Check sheet for the modelled part. Datum: model origin and axes. Units: mm. Face numbers are marked on the shaded views. A direction names the side the tool comes from. Give positions to 0.01 mm unless a question says otherwise; leave off trailing zeros. Loops run counter-clockwise (first coordinate to the right, second up) from the corner with the lowest first, then second, coordinate; pieces in that order, holes last. Notation, with made-up numbers: M 82,58.25 L 117,58.25 A26 cw 117,95.25 Z; hole C -7.75,-9.5 d10. An arc over 180 degrees is marked long. Use one line per item in the form item = value.
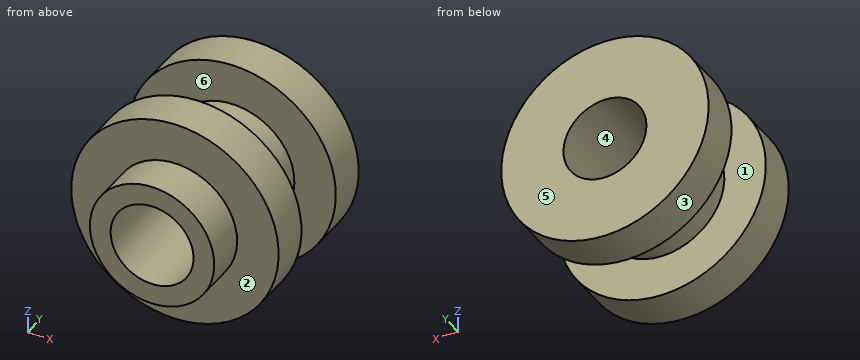
from build123d import *

# Parameters (mm, degrees)
SKETCH1_R           = 5
BOSS_EXTRUDE1_DEPTH = 9
SKETCH3_W           = 2
SKETCH3_H           = 3
SKETCH3_H_2         = 2
SKETCH4_R           = 2
CUT_EXTRUDE1_DEPTH  = 12.445523142


with BuildPart() as part:
    # Sketch1 → Boss-Extrude1 (new body)
    with BuildSketch(Plane(origin=(0, 0, 0), x_dir=(1, 0, 0), z_dir=(0, 1, 0))):
        with Locations(Location((0, 0, 0), (0, 0, 270))):
            Circle(SKETCH1_R)
    extrude(amount=BOSS_EXTRUDE1_DEPTH)

    # Sketch3 → Cut-Revolve1 (revolve, cut)
    with BuildSketch(Plane.XY, mode=Mode.PRIVATE) as cut_revolve1_sk:
        with Locations((4, 5.5)):
            Rectangle(SKETCH3_W, SKETCH3_H)
        with Locations((4, 1)):
            Rectangle(SKETCH3_W, SKETCH3_H_2)
    revolve(cut_revolve1_sk.sketch.rotate(Axis((0, 0, 0), (0, 1, 0)), 90), axis=Axis((0, 0, 0), (0, 1, 0)), mode=Mode.SUBTRACT)

    # Sketch4 → Cut-Extrude1 (cut, through all)
    with BuildSketch(Plane(origin=(0, 9, 0), x_dir=(1, 0, 0), z_dir=(0, 1, 0))):
        with Locations(Location((0, 0, 0), (0, 0, 270))):
            Circle(SKETCH4_R)
    extrude(amount=-CUT_EXTRUDE1_DEPTH, mode=Mode.SUBTRACT)


solid = part.part
1) Section check A-A (z = 0). Record the cut outline in (x, y), then the cut area to 3 significant figures.
Evaluation:
outline = M -5,2 L -3,2 L -3,0 L -2,0 L -2,9 L -5,9 L -5,7 L -3,7 L -3,4 L -5,4 Z; M 2,0 L 3,0 L 3,2 L 5,2 L 5,4 L 3,4 L 3,7 L 5,7 L 5,9 L 2,9 Z
area = 34.0 mm^2
2) Set-up check for the marked faces 1, 2 and 3: record each of +Z, -Z, +X, -X, +Y, -Y from which the full face is reachable in a straight line by a thin tool's end or side.
Evaluation:
face_1 = none
face_2 = -Y
face_3 = +Y, -Y
3) Depth check by flat-ended pin: pin 1 Ø4 at (x, y) = (1.5, 5) entering from +Z; pin 2 Ø3 at (y, z) = (1.5, 3.5) entering from -X; pin 3 Ø1 at (y, z) = (3.5, 1) entering from +X; pin 4 Ø3 at (x, z) = (0, 0) entering from +Y. Enter the tip coordinate at first touch or a pass-through.
Evaluation:
pin_1 = 5
pin_2 = -4.54
pin_3 = 4.97
pin_4 = through
4) Section check C-C (y = 6). Record the cut outline in (x, z).
Evaluation:
outline = C 0,0 d6; hole C 0,0 d4
5) Scan lines: line 1 (X direction, y = 6, z = 0); line 2 (Y direction, x = 3.25, z = 0.25); line 3 (Z direction, x = 1.5, y = 1.25). Record each from-to range of solid material in increasing order.
Evaluation:
line_1 = -3 to -2, 2 to 3
line_2 = 2 to 4, 7 to 9
line_3 = -2.6 to -1.32, 1.32 to 2.6
6) Section check B-B (x = 0). Record the cut outline in (y, z), then the cut area to 3 significant figures.
Evaluation:
outline = M 0,-3 L 2,-3 L 2,-5 L 4,-5 L 4,-3 L 7,-3 L 7,-5 L 9,-5 L 9,-2 L 0,-2 Z; M 0,2 L 9,2 L 9,5 L 7,5 L 7,3 L 4,3 L 4,5 L 2,5 L 2,3 L 0,3 Z
area = 34.0 mm^2
7) Section check D-D (z = -3.5). Record the cut outline in (x, y).
Evaluation:
outline = M -3.57,2 L 3.57,2 L 3.57,4 L -3.57,4 Z; M -3.57,7 L 3.57,7 L 3.57,9 L -3.57,9 Z
8) Release check for a two-part mould opening along Y. For the marked faces 4, 5 and 6 record: pulls with the +Y half, pulls with the -Y half, needs draft (parallel to the pull), parting line crosses it, or undercut.
Evaluation:
face_4 = needs draft
face_5 = pulls with the +Y half
face_6 = undercut
